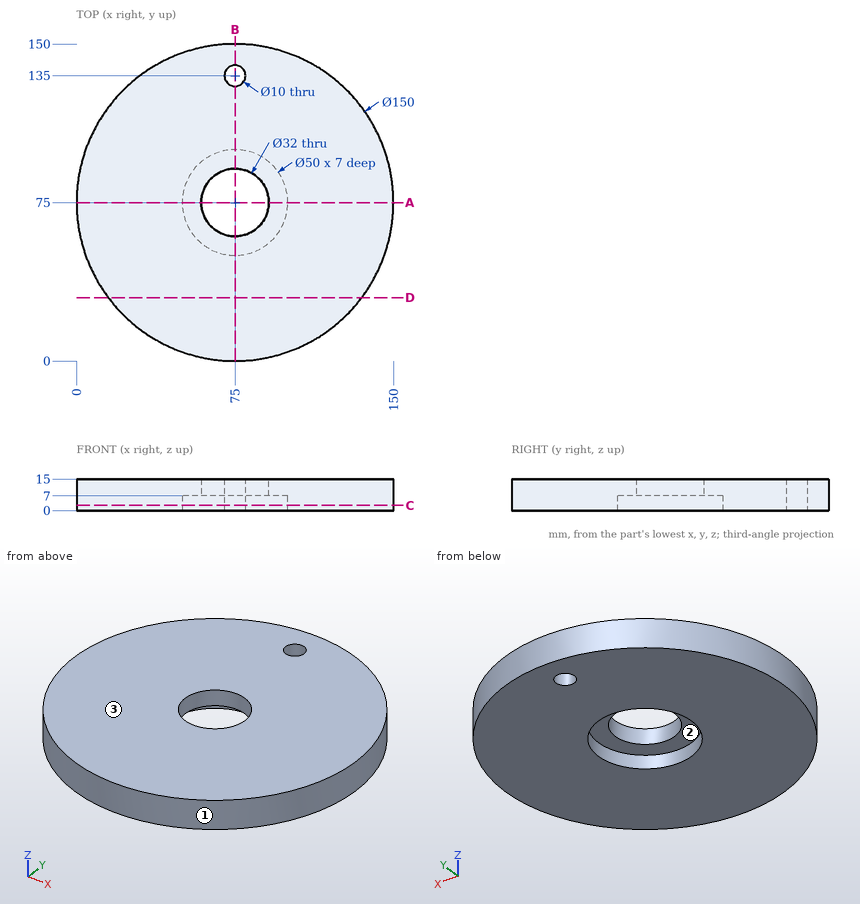
Design review of the part shown in the three views and the two pictorial views. Dimensions are in mm from the part's minimum x, y and z. Round coordinates to 2 decimals unless told otherwise and drop trailing zeros. Loops run counter-clockwise (first coordinate to the right, second up) from the corner with the lowest first, then second, coordinate; pieces in that order, holes last. Notation, with made-up numbers: (-22, 56) - (-10, 56) arc R17 cw to (-10, 72) - close; hole circle Ø7 at (34, 89). An arc over 180 degrees is marked (long way). Answer as CSV lines item,"result".
(1) Mouldability with a two-part tool opening along Y and no side actions: class the marked faces 1, 2 and 3 as +Y half, -Y half, draft (parallel to the pull), parting line (faces both ways), or undercut.
Checked values:
face 1,"parting line"
face 2,"undercut"
face 3,"draft"
(2) Consider section C-C on z = 2.5. Give the boundary of the cut face in (x, y), then the cut area to 3 significant figures.
Checked values:
outline,"circle Ø150 at (75, 75); hole circle Ø50 at (75, 75); hole circle Ø10 at (75, 135)"
area,"15,600 mm2"
(3) Wall thickness on line 1 (Y direction, x = 75, z = 10); line 2 (Y direction, x = 75, z = 2.5); line 3 (Y direction, x = 66, z = 8.25): over which ranges is each line inside the solid? List them lowest first.
Checked values:
line 1,"y = 0 to 59, 91 to 130, 140 to 150"
line 2,"y = 0 to 50, 100 to 130, 140 to 150"
line 3,"y = 0.54 to 61.77, 88.23 to 149.46"
(4) Consider section D-D on y = 30. Give the boundary of the cut face in (x, z).
Checked values:
outline,"(15, 0) - (135, 0) - (135, 15) - (15, 15) - close"
(5) Insertion check: P1, Ø5, axis at x = 19, y = 131, coming from the -Z side; P2, Ø5, axis at y = 132, z = 4, coming from the -X side; P3, Ø1, axis at x = 79.5, z = 12.5, coming from the +Y side; P4, Ø15, axis at x = 63.5, y = 79.5, coming from the -Z side. Each pin has a flat end and moves straight along its axis. Give the tip position at first contact, or say it passes through.
Checked values:
P1,"passes through"
P2,"stops at x = 23.48"
P3,"stops at y = 149.89"
P4,"stops at z = 7"
(6) Consider section B-B on x = 75. Give the boundary of the cut face in (y, z).
Checked values:
outline,"(0, 0) - (50, 0) - (50, 7) - (59, 7) - (59, 15) - (0, 15) - close; (91, 7) - (100, 7) - (100, 0) - (130, 0) - (130, 15) - (91, 15) - close; (140, 0) - (150, 0) - (150, 15) - (140, 15) - close"
(7) Consider section A-A on y = 75. Give the boundary of the cut face in (x, z), then the cut area to 3 significant figures.
Checked values:
outline,"(0, 0) - (50, 0) - (50, 7) - (59, 7) - (59, 15) - (0, 15) - close; (91, 7) - (100, 7) - (100, 0) - (150, 0) - (150, 15) - (91, 15) - close"
area,"1,640 mm2"
